Design review of the part built by this model. Coordinates are the model's own, in mm. Coordinates: 2 decimals unless noted, no trailing zeros. Loops run counter-clockwise (first coordinate to the right, second up) from the corner with the lowest first, then second, coordinate; pieces in that order, holes last. Notation, with made-up numbers: (82, 63) -> (89, 63) arc R8 ccw to (89, 67) -> close; hole circle Ø7 at (-16, -25). An arc over 180 degrees is marked (long way). One line per item, written item: value. Start each with the question number.
1. Add section A-A on y = 112.5. Write out the cut boundary in (x, z), plus the area to 3 significant figures.
2. Add section C-C on x = 100. Write out the cut boundary in (y, z).
3. For probe 1 along Z at (x, y) = (-70, 160); probe 2 along Y at (x, z) = (-67, -22.5); probe 3 along X at (y, z) = (147, 0), list the stretches that pass through material, from the lowest coordinate up.
4. Insertion check: pin 1 (6 mm diameter, centred on y = 116, z = 15.5, fed in from +X); pin 2 (12 mm diameter, centred on x = 37.5, z = -14.5, fed in from +Y); pin 3 (5 mm diameter, centred on y = 53, z = -19, fed in from +X). Each pin has a flat end and moves straight along its axis. Give the tip position at first contact, or say it passes through.
5. Draft analysis for pull direction Z (two halves, no side actions). For faces 1 (the flat face through (-71.84, 159.29, -24.32)), 2 (the flat face through (-73.37, 159.29, 24.21)), 3 (the cylindrical face through (-72.449, 159.979, 9.696)), state which applies: pulls with the +Z half, pulls with the -Z half, needs draft (parallel to the pull), parting line crosses it, or undercut.
6. Add section B-B on z = 0. Write out the cut boundary in (x, y), plus the area to 3 significant figures.
7. Add section D-D on x = -32. Write out the cut boundary in (y, z).
```python
from build123d import *

# Parameters (mm, degrees)
SHEET_EXTRUDE_1_1_BACK   = 40
SHEET_EXTRUDE_1_1_DEPTH  = 80
THICKEN_1_T1             = 1
THICKEN_1_T2             = 1
SKETCH_2_OUTSIDE_W       = 406.64
SKETCH_2_OUTSIDE_H       = 158.22
CUT_EXTRUDE_1_DEPTH      = 253.095220105
CUT_EXTRUDE_2_REACH      = 254.095
CUT_EXTRUDE_2_END_RADIUS = 176
SKETCH_3_W               = 40
SKETCH_3_H               = 17
CUT_EXTRUDE_3_REACH      = 254.095
CUT_EXTRUDE_3_END_RADIUS = 176
SKETCH_4_R               = 20
CUT_EXTRUDE_4_REACH      = 254.095
SKETCH_5_R               = 10


with BuildPart() as body_1:
    # Sheet Extrude 1: a surface, the sketch's curves swept straight by 80 mm
    with BuildLine(Plane.XY.offset(-SHEET_EXTRUDE_1_1_BACK), mode=Mode.PRIVATE) as sheet_extrude_1_1_path:
        ThreePointArc((151.554445662, 87.5), (-45.293332893, 169.037019601), (-175, 0))
    sheet_extrude_1_1 = Shell.extrude(sheet_extrude_1_1_path.wire(), (0 * SHEET_EXTRUDE_1_1_DEPTH, 0 * SHEET_EXTRUDE_1_1_DEPTH, 1 * SHEET_EXTRUDE_1_1_DEPTH))
    add(Solid.thicken(sheet_extrude_1_1, THICKEN_1_T1))
    add(Solid.thicken(sheet_extrude_1_1, -THICKEN_1_T2))

    # 草图2 outside → 切除-拉伸1 (cut, through all)
    with BuildSketch(Plane(origin=(0, 0, 0), x_dir=(1, 0, 0), z_dir=(0, 1, 0))):
        with Locations((-11.79, 0)):
            Rectangle(SKETCH_2_OUTSIDE_W, SKETCH_2_OUTSIDE_H)
        Polygon((152.420471066, 40), (-197.579528934, 15.52561582), (-197.579528934, -15.52561582), (152.420471066, -40), align=None, mode=Mode.SUBTRACT)
    extrude(amount=CUT_EXTRUDE_1_DEPTH, mode=Mode.SUBTRACT)

    # 切除-拉伸2: up to this cylinder (the profile starts inside it)
    cut_extrude_2_end = Plane(origin=(0, 0, 0), z_dir=(0, 0, 1)) * Cylinder(CUT_EXTRUDE_2_END_RADIUS, 861.19, mode=Mode.PRIVATE)
    # 草图3 → 切除-拉伸2 (cut, up to the surface)
    with BuildSketch(Plane(origin=(0, 0, 0), x_dir=(1, 0, 0), z_dir=(0, 1, 0)), mode=Mode.PRIVATE) as cut_extrude_2_sk1:
        Rectangle(SKETCH_3_W, SKETCH_3_H)
    cut_extrude_2_tool1 = extrude(cut_extrude_2_sk1.sketch, amount=CUT_EXTRUDE_2_REACH, mode=Mode.PRIVATE) & cut_extrude_2_end
    add(cut_extrude_2_tool1.solids().sort_by_distance((0, 0, 0))[0], mode=Mode.SUBTRACT)

    # 切除-拉伸3: up to this cylinder (the profile starts inside it)
    cut_extrude_3_end = Plane(origin=(0, 0, 0), z_dir=(0, 0, 1)) * Cylinder(CUT_EXTRUDE_3_END_RADIUS, 861.19, mode=Mode.PRIVATE)
    # 草图4 → 切除-拉伸3 (cut, up to the surface)
    with BuildSketch(Plane(origin=(0, 0, 0), x_dir=(1, 0, 0), z_dir=(0, 1, 0)), mode=Mode.PRIVATE) as cut_extrude_3_sk1:
        with Locations(Location((100, 0, 0), (0, 0, 90))):
            Circle(SKETCH_4_R)
    cut_extrude_3_tool1 = extrude(cut_extrude_3_sk1.sketch, amount=CUT_EXTRUDE_3_REACH, mode=Mode.PRIVATE) & cut_extrude_3_end
    add(cut_extrude_3_tool1.solids().sort_by_distance((100, 0, 0))[0], mode=Mode.SUBTRACT)

    # 草图5 → 切除-拉伸4 (cut, up to next)
    with BuildSketch(Plane(origin=(0, 0, 0), x_dir=(1, 0, 0), z_dir=(0, 1, 0)), mode=Mode.PRIVATE) as cut_extrude_4_sk1:
        with Locations(Location((-70, 0, 0), (0, 0, 90))):
            Circle(SKETCH_5_R)
    cut_extrude_4_tool1 = extrude(cut_extrude_4_sk1.sketch, amount=CUT_EXTRUDE_4_REACH, mode=Mode.PRIVATE) & body_1.part
    add(cut_extrude_4_tool1.solids().sort_by_distance((-70, 0, 0))[0], mode=Mode.SUBTRACT)


solid = body_1.part
```
Worked answers:
1. outline: (-135.35, -19.88) -> (-132.74, -20.06) -> (-132.74, 20.06) -> (-135.35, 19.88) -> close; (132.74, -38.62) -> (135.35, -38.81) -> (135.35, 38.81) -> (132.74, 38.62) -> close
1. area: 306 mm²
2. outline: (142.39, -36.33) -> (144.83, -36.33) -> (144.83, -20) -> (142.39, -20) -> close; (142.39, 20) -> (144.83, 20) -> (144.83, 36.33) -> (142.39, 36.33) -> close
3. probe 1: z = -24.45 to -10, 10 to 24.45
3. probe 2: y = 160.58 to 162.75
3. probe 3: x = -96.78 to -93.1
4. pin 1: stops at x = 134.93
4. pin 2: stops at y = 173.16
4. pin 3: stops at x = -165.01
5. face 1: pulls with the -Z half
5. face 2: pulls with the +Z half
5. face 3: undercut
6. outline: (-176, 0) -> (-174, 0) arc R174 cw to (-80, 154.52) -> (-80, 156.77) arc R176 ccw to start; (-60, 163.33) arc R174 cw to (-20, 172.85) -> (-20, 174.86) arc R176 ccw to (-60, 165.46) -> close; (20, 172.85) arc R174 cw to (80, 154.52) -> (80, 156.77) arc R176 ccw to (20, 174.86) -> close; (120, 126) arc R174 cw to (150.69, 87) -> (152.42, 88) arc R176 ccw to (120, 128.75) -> close
6. area: 694 mm²
7. outline: (171.03, -27.1) -> (173.07, -27.1) -> (173.07, 27.1) -> (171.03, 27.1) -> close
